```python
from build123d import *

# Parameters (mm, degrees)
CHAMFER2_SIZE                      = 0.762
CHAMFER2_SIZE2                     = 0.439940905
CHAMFER3_SIZE                      = 1.524
F_1_8_NPT_TAPPED_HOLE1_D           = 8.4328
F_1_8_NPT_TAPPED_HOLE1_DEPTH       = 63.119
F_1_8_NPT_TAPPED_HOLE1_CBORE_D     = 12.5731524
F_1_8_NPT_TAPPED_HOLE1_CBORE_DEPTH = 58.42
F_1_8_NPT_TAPPED_HOLE1_TIP         = 2.533468714


with BuildPart() as part:
    # Sketch1 → Revolve1 (revolve)
    with BuildSketch(Plane.XY, mode=Mode.PRIVATE) as revolve1_sk:
        with BuildLine():
            Line((0, 101.6), (41.402, 101.6))
            Line((41.402, 101.6), (41.402, 88.011))
            ThreePointArc((41.402, 88.011), (40.955630735, 86.933369265), (39.878, 86.487))
            Line((39.878, 86.487), (37.400925561, 86.487))
            Line((37.400925561, 86.487), (35.884220112, 86.8934))
            ThreePointArc((35.884220112, 86.8934), (35.223123791, 86.761899766), (34.925, 86.15736452))
            Line((34.925, 86.15736452), (34.925, 80.899))
            ThreePointArc((34.925, 80.899), (34.701815367, 80.360184633), (34.163, 80.137))
            Line((34.163, 80.137), (29.293607942, 80.137))
            ThreePointArc((29.293607942, 80.137), (29.096387829, 80.11103548), (28.912607942, 80.034911358))
            Line((28.912607942, 80.034911358), (26.516622715, 78.651588642))
            ThreePointArc((26.516622715, 78.651588642), (26.332842828, 78.57546452), (26.135622715, 78.5495))
            Line((26.135622715, 78.5495), (0, 78.5495))
            Line((0, 78.5495), (0, 101.6))
        make_face()
    revolve(revolve1_sk.sketch.rotate(Axis((-48.080119454, 0, 0), (1, 0, 0)), 90), axis=Axis((-48.080119454, 0, 0), (1, 0, 0)))

    # Chamfer2
    chamfer2_edges = [part.edges().sort_by_distance(p)[0] for p in [
        (0, 0, -78.5495),
    ]]
    chamfer2_side = [part.faces().sort_by_distance(p)[0] for p in [
        (13.067811358, 0, -78.5495),
    ]]
    chamfer(chamfer2_edges, length=CHAMFER2_SIZE, length2=CHAMFER2_SIZE2, reference=chamfer2_side[0])

    # Chamfer3
    chamfer3_edges = [part.edges().sort_by_distance(p)[0] for p in [
        (41.402, 0, -101.6),
        (0, 0, -101.6),
    ]]
    chamfer(chamfer3_edges, length=CHAMFER3_SIZE)

    # 1/8 NPT Tapped Hole1
    with Locations(Plane(origin=(26.3144, 101.6, 0), x_dir=(0, 0, 1), z_dir=(0, 1, 0))):
        with Locations((0, 0)):
            CounterBoreHole(F_1_8_NPT_TAPPED_HOLE1_D / 2, F_1_8_NPT_TAPPED_HOLE1_CBORE_D / 2, F_1_8_NPT_TAPPED_HOLE1_CBORE_DEPTH, depth=F_1_8_NPT_TAPPED_HOLE1_DEPTH)
            with Locations((0, 0, -(F_1_8_NPT_TAPPED_HOLE1_DEPTH + F_1_8_NPT_TAPPED_HOLE1_TIP / 2))):  # 118° drill point
                Cone(0, F_1_8_NPT_TAPPED_HOLE1_D / 2, F_1_8_NPT_TAPPED_HOLE1_TIP, mode=Mode.SUBTRACT)


solid = part.part
```
Source: CAD feature listing. Evaluate the final solid. Frame: model axes, mm. A direction names the side the tool comes from. Give positions to 0.01 mm unless a question says otherwise; leave off trailing zeros. Loops run counter-clockwise (first coordinate to the right, second up) from the corner with the lowest first, then second, coordinate; pieces in that order, holes last. Notation, with made-up numbers: (15, -35.75) -> (31, -35.75) arc R30 cw to (31, 1.25) -> close; hole circle Ø5 at (70, 21.25). An arc over 180 degrees is marked (long way). Put each result on its own line as item: value. Start each with the question number.
1) Reachability of faces 5 (the face through (31.694, -24.071, 76.436)), 6 (the face through (0, -30, -74)) from +Z, -Z, +X, -X, +Y, -Y: full face, straight path, thin tool, end or side. Return the list, or none.
2) Draft query along Z for faces 1 (the face through (20.97, 61.82, -80.63)), 2 (the face through (20.177, 90.114, -1.363)), 3 (the face through (41.402, 88.5, -0.5)), 4 (the face through (13.27, -77.88, -10.23)). Return one class per face: released by +Z, released by -Z, zero draft, split by the parting line, or undercut.
3) Contact query for flat-ended pins moving along their axis: P1, Ø3, axis at x = 27, y = -55.5, coming from the +Z side; P2, Ø1, axis at x = 22.5, y = -78, coming from the -Z side; P3, Ø5, axis at x = 9, z = -65, coming from the -Y side. Output: stop coordinate, or through.
4) Cut plane A-A (z = 0). State how many separate pieces and enclosed holes the cut face has, then the cut area to 3 significant figures.
5) Material intervals for probe 1 along Y at (x, z) = (19.5, 0); probe 2 along Y at (x, z) = (39.35, 0), sorted ascending.
6) Cut plane B-B (x = 16.5). Return loops of the section in (y, z), then the cut area to 3 significant figures.
Results are:
1. face 5: +X
1. face 6: +Z, -Z, -X, +Y, -Y
2. face 1: split by the parting line
2. face 2: undercut
2. face 3: zero draft
2. face 4: undercut
3. P1: stops at z = 86.06
3. P2: stops at z = -65.7
3. P3: stops at y = -80.1
4. separate pieces: 3
4. enclosed holes: 0
4. area: 1,490 mm2
5. probe 1: y = -101.6 to -78.55, 78.55 to 101.6
5. probe 2: y = -101.6 to -86.49, 86.49 to 101.6
6. outline: circle Ø203.2 at (0, 0); hole circle Ø157.1 at (0, 0)
6. area: 13,000 mm2
